```python
from build123d import *

# Parameters (mm, degrees)
SKETCH_1_R        = 10
SKETCH_1_R_2      = 8
EXTRUDE_1_DEPTH   = 11
SKETCH_2_R        = 5
EXTRUDE_1_2_DEPTH = 10
SKETCH_3_R        = 7
SKETCH_3_R_2      = 5
EXTRUDE_2_DEPTH   = 10


with BuildPart() as part:
    # 草图1 → Extrude 1 (new body)
    with BuildSketch(Plane(origin=(0, 0, 0), x_dir=(1, 0, 0), z_dir=(0, 1, 0))):
        Circle(SKETCH_1_R)
        Circle(SKETCH_1_R_2, mode=Mode.SUBTRACT)
    extrude(amount=EXTRUDE_1_DEPTH)

    # 草图2 → Extrude 1 2 (add)
    with BuildSketch(Plane.XZ):
        Polygon((11.547005384, 0), (5.773502692, 10), (-5.773502692, 10), (-11.547005384, 0), (-5.773502692, -10), (5.773502692, -10), align=None)
        with Locations(Location((0, 0, 0), (0, 0, 270))):
            Circle(SKETCH_2_R, mode=Mode.SUBTRACT)
    extrude(amount=EXTRUDE_1_2_DEPTH)

    # 草图3 → 拉伸-薄壁2 (add)
    with BuildSketch(Plane.XZ.offset(10)):
        Circle(SKETCH_3_R)
        Circle(SKETCH_3_R_2, mode=Mode.SUBTRACT)
    extrude(amount=EXTRUDE_2_DEPTH)


solid = part.part
```
CAD build for the part. Positions are in the model's coordinates, mm. A direction names the side the tool comes from. Coordinates: 2 decimals unless noted, no trailing zeros. Write each loop counter-clockwise with the first axis right and the second up, starting at its lowest first coordinate (ties: lowest second). Pieces come first, ordered by that corner, then holes.
(1) Flat gauge pins, fed straight in: pin 1 (5 mm diameter, centred on y = -0.5, z = -7, fed in from +X); pin 2 (4 mm diameter, centred on x = 8.5, z = -3.5, fed in from -Y); pin 3 (1 mm diameter, centred on x = 7.5, z = 7.5, fed in from +Y); pin 4 (6 mm diameter, centred on x = 0, z = 0, fed in from -Y). Where does each tip first touch, or does it go through?
(2) 3-axis set-ups, long thin cutter, end or side, ignore diameter. For faces 4 (the face through (-2.17, 5.42, 9.76)), 5 (the face through (5, 0, 9)), 6 (the face through (2, -10, 7)): which of +Z, -Z, +X, -X, +Y, -Y reach the whole face in a straight line?
(3) Cut at C-C, the plane x = 6.5. List the corners of the cut face in (y, z), and give its area (3 significant figures).
(4) Drill centre lines: probe 1 along X at (y, z) = (-7, 0); probe 2 along Z at (x, y) = (0, -5.5); probe 3 along Z at (x, y) = (0, 4.25). Where is each one in solid material? Low to high.
(5) Cut at A-A, the plane y = -1.5. List the corners of the cut face in (x, z).
(6) Cut at B-B, the plane z = 0.5. List the corners of the cut face in (x, y).
(7) Two-plate mould, pull along Y, no slides. Class faces 1 (the face through (-10.3, 0, 0)), 2 (the face through (-8.62, -4.93, 5.07)), 3 (the face through (-2, -20, 5)): +Y half, -Y half, draft (parallel to the pull), parting line (faces both ways), or undercut.
Geometry says:
1. pin 1: stops at x = 8.95
1. pin 2: stops at y = -10
1. pin 3: stops at y = 0
1. pin 4: passes through
2. face 4: +Y
2. face 5: +Z, +X, +Y
2. face 6: -Y
3. outline: (-20, -2.6) - (-10, -2.6) - (-10, -8.74) - (0, -8.74) - (0, -7.6) - (11, -7.6) - (11, -4.66) - (0, -4.66) - (0, 4.66) - (11, 4.66) - (11, 7.6) - (0, 7.6) - (0, 8.74) - (-10, 8.74) - (-10, 2.6) - (-20, 2.6) - close
3. area: 291 mm2
4. probe 1: x = -11.55 to -5, 5 to 11.55
4. probe 2: z = -10 to -5, 5 to 10
4. probe 3: z = -10 to -8, 8 to 10
5. outline: (-11.55, 0) - (-5.77, -10) - (5.77, -10) - (11.55, 0) - (5.77, 10) - (-5.77, 10) - close; hole circle Ø10 at (0, 0)
6. outline: (-11.26, -10) - (-6.98, -10) - (-6.98, -20) - (-4.97, -20) - (-4.97, 0) - (-7.98, 0) - (-7.98, 11) - (-9.99, 11) - (-9.99, 0) - (-11.26, 0) - close; (4.97, -20) - (6.98, -20) - (6.98, -10) - (11.26, -10) - (11.26, 0) - (9.99, 0) - (9.99, 11) - (7.98, 11) - (7.98, 0) - (4.97, 0) - close
7. face 1: +Y half
7. face 2: draft
7. face 3: -Y half
